Work out the finished part from the listing and answer in its coordinate system (mm). Give positions to 0.01 mm unless a question says otherwise; leave off trailing zeros. Loops run counter-clockwise (first coordinate to the right, second up) from the corner with the lowest first, then second, coordinate; pieces in that order, holes last. Notation, with made-up numbers: (1, -35) - (28, -35) arc R17 ccw to (28, -6) - close; hole circle Ø7 at (-34.5, 63). An arc over 180 degrees is marked (long way). Use CSV: the item, a comma, the result in double quotes.
from build123d import *

# Parameters (mm, degrees)
BOSS_EXTRUDE1_DEPTH = 33


with BuildPart() as part:
    # Sketch1 → Boss-Extrude1 (new body)
    with BuildSketch(Plane(origin=(33, 0, 0), x_dir=(0, 0, -1), z_dir=(1, 0, 0))):
        with BuildLine():
            ThreePointArc((20.995176507, 0.450070465), (17.237696927, 2.548883943), (12.962492698, 2.05259812))
            ThreePointArc((12.962492698, 2.05259812), (12.48166572, 4.055539034), (11.693363786, 5.958575279))
            ThreePointArc((11.693363786, 5.958575279), (15.443786149, 8.06997361), (17.249999376, 11.976540465))
            ThreePointArc((17.249999376, 11.976540465), (16.989356882, 12.343490298), (16.720909812, 12.704769776))
            ThreePointArc((16.720909812, 12.704769776), (12.447393366, 12.194154464), (9.280389979, 9.279748803))
            ThreePointArc((9.280389979, 9.279748803), (7.714093651, 10.617539034), (5.957767351, 11.693775447))
            ThreePointArc((5.957767351, 11.693775447), (7.750873978, 15.606375533), (6.91590879, 19.828520006))
            ThreePointArc((6.91590879, 19.828520006), (6.489356882, 19.972186842), (6.059823892, 20.106678851))
            ThreePointArc((6.059823892, 20.106678851), (2.902608611, 17.181672443), (2.053493716, 12.96235085))
            ThreePointArc((2.053493716, 12.96235085), (0, 13.124), (-2.053493716, 12.96235085))
            ThreePointArc((-2.053493716, 12.96235085), (-2.902608611, 17.181672443), (-6.059823892, 20.106678851))
            ThreePointArc((-6.059823892, 20.106678851), (-6.489356882, 19.972186842), (-6.91590879, 19.828520006))
            ThreePointArc((-6.91590879, 19.828520006), (-7.750873978, 15.606375533), (-5.957767351, 11.693775447))
            ThreePointArc((-5.957767351, 11.693775447), (-7.714093651, 10.617539034), (-9.280389979, 9.279748803))
            ThreePointArc((-9.280389979, 9.279748803), (-12.447393366, 12.194154464), (-16.720909812, 12.704769776))
            ThreePointArc((-16.720909812, 12.704769776), (-16.989356882, 12.343490298), (-17.249999376, 11.976540465))
            ThreePointArc((-17.249999376, 11.976540465), (-15.443786149, 8.06997361), (-11.693363786, 5.958575279))
            ThreePointArc((-11.693363786, 5.958575279), (-12.48166572, 4.055539034), (-12.962492698, 2.05259812))
            ThreePointArc((-12.962492698, 2.05259812), (-17.237696927, 2.548883943), (-20.995176507, 0.450070465))
            ThreePointArc((-20.995176507, 0.450070465), (-21, 0), (-20.995176507, -0.450070465))
            ThreePointArc((-20.995176507, -0.450070465), (-17.237696927, -2.548883943), (-12.962492698, -2.05259812))
            ThreePointArc((-12.962492698, -2.05259812), (-12.48166572, -4.055539034), (-11.693363786, -5.958575279))
            ThreePointArc((-11.693363786, -5.958575279), (-15.443786149, -8.06997361), (-17.249999376, -11.976540465))
            ThreePointArc((-17.249999376, -11.976540465), (-16.989356882, -12.343490298), (-16.720909812, -12.704769776))
            ThreePointArc((-16.720909812, -12.704769776), (-12.447393366, -12.194154464), (-9.280389979, -9.279748803))
            ThreePointArc((-9.280389979, -9.279748803), (-7.714093651, -10.617539034), (-5.957767351, -11.693775447))
            ThreePointArc((-5.957767351, -11.693775447), (-7.750873978, -15.606375533), (-6.91590879, -19.828520006))
            ThreePointArc((-6.91590879, -19.828520006), (-6.489356882, -19.972186842), (-6.059823892, -20.106678851))
            ThreePointArc((-6.059823892, -20.106678851), (-2.902608611, -17.181672443), (-2.053493716, -12.96235085))
            ThreePointArc((-2.053493716, -12.96235085), (0, -13.124), (2.053493716, -12.96235085))
            ThreePointArc((2.053493716, -12.96235085), (2.902608611, -17.181672443), (6.059823892, -20.106678851))
            ThreePointArc((6.059823892, -20.106678851), (6.489356882, -19.972186842), (6.91590879, -19.828520006))
            ThreePointArc((6.91590879, -19.828520006), (7.750873978, -15.606375533), (5.957767351, -11.693775447))
            ThreePointArc((5.957767351, -11.693775447), (7.714093651, -10.617539034), (9.280389979, -9.279748803))
            ThreePointArc((9.280389979, -9.279748803), (12.447393366, -12.194154464), (16.720909812, -12.704769776))
            ThreePointArc((16.720909812, -12.704769776), (16.989356882, -12.343490298), (17.249999376, -11.976540465))
            ThreePointArc((17.249999376, -11.976540465), (15.443786149, -8.06997361), (11.693363786, -5.958575279))
            ThreePointArc((11.693363786, -5.958575279), (12.48166572, -4.055539034), (12.962492698, -2.05259812))
            ThreePointArc((12.962492698, -2.05259812), (17.237696927, -2.548883943), (20.995176507, -0.450070465))
            ThreePointArc((20.995176507, -0.450070465), (21, 0), (20.995176507, 0.450070465))
        make_face()
        with BuildLine():
            Line((2.5, 10.3), (2.5, 7.599342077))
            ThreePointArc((2.5, 7.599342077), (0, -8), (-2.5, 7.599342077))
            Line((-2.5, 7.599342077), (-2.5, 10.3))
            Line((-2.5, 10.3), (2.5, 10.3))
        make_face(mode=Mode.SUBTRACT)
    extrude(amount=-BOSS_EXTRUDE1_DEPTH)


solid = part.part
Item 1: A cutting plane is placed at D-D on z = 18. Determine the outline of the cut face in (x, y), and give its area (3 significant figures).
Determined:
outline,"(0, -2.35) - (33, -2.35) - (33, 2.35) - (0, 2.35) - close"
area,"155 mm²"
Item 2: Find the intervals of material crossed by line 1 (Z direction, x = 13, y = 0); line 2 (Y direction, x = 19, z = 0); line 3 (Z direction, x = 30.5, y = -12), in increasing order.
Determined:
line 1,"z = -21 to -8, 8 to 21"
line 2,"y = -13.12 to -8, 10.3 to 13.12"
line 3,"z = -17.23 to -12.06, -6.22 to 6.22, 12.06 to 17.23"
Item 3: Given P1, Ø2, axis at y = -7.5, z = 1, coming from the -X side; P2, Ø1.5, axis at x = 12, y = 10, coming from the +Z side; P3, Ø0.8, axis at x = 13, y = 8.5, coming from the +Z side; P4, Ø1.4, axis at x = 15, y = 9.5, coming from the -Z side, each flat-ended and moving along its own axis, determine where each tip first touches the part or whether it passes through.
Determined:
P1,"stops at x = 0"
P2,"stops at z = 16.99"
P3,"stops at z = 16.1"
P4,"stops at z = -16.79"
Item 4: A cutting plane is placed at A-A on z = 0. Determine the outline of the cut face in (x, y), and give its area (3 significant figures).
Determined:
outline,"(0, -13.12) - (33, -13.12) - (33, -8) - (0, -8) - close; (0, 10.3) - (33, 10.3) - (33, 13.12) - (0, 13.12) - close"
area,"262 mm²"
Item 5: A cutting plane is placed at B-B on y = 4.5. Determine the outline of the cut face in (x, z).
Determined:
outline,"(0, -12.33) - (33, -12.33) - (33, -6.61) - (0, -6.61) - close; (0, 6.61) - (33, 6.61) - (33, 12.33) - (0, 12.33) - close"
Item 6: A cutting plane is placed at C-C on z = -11. Determine the outline of the cut face in (x, y).
Determined:
outline,"(0, -11.3) - (33, -11.3) - (33, 11.3) - (0, 11.3) - close"
Item 7: The mould has two halves that part along Y. Classify faces 1 (the flat face through (0, -9, 0)), 2 (the cylindrical face through (16.731, -10.634, -7.691)): pulls with the +Y half, pulls with the -Y half, needs draft (parallel to the pull), parting line crosses it, or undercut.
Determined:
face 1,"needs draft"
face 2,"undercut"
